```python
from build123d import *

# Parameters (mm, degrees)
SKETCH_2_R          = 30
EXTRUDE_1_DEPTH     = 470
CUT_EXTRUDE_START   = -25
SKETCH_3_R          = 30
SKETCH_3_R_2        = 20
CUT_EXTRUDE_1_DEPTH = 25
SKETCH_4_R          = 30
SKETCH_4_R_2        = 20
CUT_EXTRUDE_2_DEPTH = 25
SKETCH_5_W          = 6
SKETCH_5_H          = 220


with BuildPart() as part:
    # 草图2 → 凸台-拉伸1 (new body)
    with BuildSketch(Plane.XY):
        with Locations(Location((0, 0, 0), (0, 0, 180))):
            Circle(SKETCH_2_R)
    extrude(amount=EXTRUDE_1_DEPTH)

    # 草图3 → 切除-拉伸1 (cut)
    with BuildSketch(Plane.XY.offset(470).offset(CUT_EXTRUDE_START)):
        with Locations(Location((0, 0, 0), (0, 0, 180))):
            Circle(SKETCH_3_R)
        Circle(SKETCH_3_R_2, mode=Mode.SUBTRACT)
    extrude(amount=CUT_EXTRUDE_1_DEPTH, mode=Mode.SUBTRACT)

    # 草图4 → 切除-拉伸2 (cut)
    with BuildSketch(Plane(origin=(0, 0, 0), x_dir=(-1, 0, 0), z_dir=(0, 0, -1))):
        Circle(SKETCH_4_R)
        with Locations(Location((0, 0, 0), (0, 0, 180))):
            Circle(SKETCH_4_R_2, mode=Mode.SUBTRACT)
    extrude(amount=-CUT_EXTRUDE_2_DEPTH, mode=Mode.SUBTRACT)

    # 草图5 → 切除-旋转1 (revolve, cut)
    with BuildSketch(Plane(origin=(0, 0, 0), x_dir=(1, 0, 0), z_dir=(0, 1, 0))):
        with Locations((-27, -235)):
            Rectangle(SKETCH_5_W, SKETCH_5_H)
    revolve(axis=Axis((0, 0, 345), (0, 0, -1)), mode=Mode.SUBTRACT)

    # 草图6 → 切除-旋转2 (revolve, cut)
    with BuildSketch(Plane(origin=(0, 0, 0), x_dir=(1, 0, 0), z_dir=(0, 1, 0))):
        Polygon((20, -470), (19, -470), (20, -469), align=None)
        Polygon((20, -1), (19, 0), (20, 0), align=None)
    revolve(axis=Axis((0, 0, 470), (0, 0, -1)), mode=Mode.SUBTRACT)


solid = part.part
```
Can you work these out from the model? Positions are in its coordinate system, mm. A direction names the side the tool comes from. Coordinates: 2 decimals unless noted, no trailing zeros. Loops run counter-clockwise (first coordinate to the right, second up) from the corner with the lowest first, then second, coordinate; pieces in that order, holes last.
Item 1: If we mould it in two halves opening along Z, with no side actions, what happens to faces 4 (the face through (0, 0, 0)), 5 (the face through (-6, 20, 445)), 6 (the face through (23.977, 1.055, 233.46)), 7 (the face through (-16.128, -25.296, 394.3))? For each: released by +Z, released by -Z, zero draft, split by the parting line, or undercut.
Answers below:
face 4: released by -Z
face 5: released by +Z
face 6: undercut
face 7: zero draft
Item 2: Suppose I cut it at A-A (y = 0). Please give me the cut outline in (x, z), then the cut area to 3 significant figures.
Answers below:
outline: (-30, 25) - (-20, 25) - (-20, 1) - (-19, 0) - (19, 0) - (20, 1) - (20, 25) - (30, 25) - (30, 125) - (24, 125) - (24, 345) - (30, 345) - (30, 445) - (20, 445) - (20, 469) - (19, 470) - (-19, 470) - (-20, 469) - (-20, 445) - (-30, 445) - (-30, 345) - (-24, 345) - (-24, 125) - (-30, 125) - close
area: 24,600 mm2
Item 3: I'm going to push flat-ended pins straight in: pin 1 (1.5 mm diameter, centred on x = -20, y = 11, fed in from -Z); pin 2 (4 mm diameter, centred on y = -9, z = 102.5, fed in from +X); pin 3 (12 mm diameter, centred on y = -9.5, z = 276.5, fed in from -X). Where does each tip first touch, or does it pass through?
Answers below:
pin 1: stops at z = 25
pin 2: stops at x = 29.17
pin 3: stops at x = -23.74
Item 4: Suppose I cut it at C-C (z = 171). Please give me the cut outline in (x, y), then the cut area to 3 significant figures.
Answers below:
outline: circle Ø48 at (0, 0)
area: 1,810 mm2
Item 5: Please list where these lines run through material, in increasing order: L1, parallel to Z at x = -25, y = 7; L2, parallel to Z at x = -21.5, y = 5.5; L3, parallel to X at y = -1, z = 136.
Answers below:
L1: z = 25 to 125, 345 to 445
L2: z = 25 to 445
L3: x = -23.98 to 23.98
Item 6: Which directions (+Z, -Z, +X, -X, +Y, -Y) give clear straight access to the entire face, cutting with the end or side of a thin tool? Please do faces 1 (the face through (-4.336, -19.524, 456.832)), 2 (the face through (-19.98, -0.88, 12.83)), 3 (the face through (13.5, 20.1, 125)).
Answers below:
face 1: +Z
face 2: -Z
face 3: none
